from build123d import *

# Parameters (mm, degrees)
SKETCH_1_W          = 40
SKETCH_1_H          = 20
SKETCH_1_R          = 2.25
EXTRUDE_1_DEPTH     = 10
SKETCH_3_R          = 1.65
CUT_EXTRUDE_1_DEPTH = 11.5
CUT_EXTRUDE_START   = -11.5
SKETCH_4_R          = 1.65
CUT_EXTRUDE_2_DEPTH = 11.5


with BuildPart() as part:
    # 草图1 → 凸台-拉伸1 (new body)
    with BuildSketch(Plane.XY):
        with Locations((0.651465798, 0.195439739)):
            Rectangle(SKETCH_1_W, SKETCH_1_H)
        with Locations((-9.348534202, 0.195439739)):
            Circle(SKETCH_1_R, mode=Mode.SUBTRACT)
        with Locations((10.651465798, 0.195439739)):
            Circle(SKETCH_1_R, mode=Mode.SUBTRACT)
    extrude(amount=EXTRUDE_1_DEPTH)

    # 草图3 → 切除-拉伸1 (cut)
    with BuildSketch(Plane.ZY.offset(19.348534202)):
        with Locations(Location((5, 4.195439739, 0), (0, 0, 270))):
            Circle(SKETCH_3_R)
        with Locations(Location((5, -3.804560261, 0), (0, 0, 270))):
            Circle(SKETCH_3_R)
    extrude(amount=-CUT_EXTRUDE_1_DEPTH, mode=Mode.SUBTRACT)

    # 草图4 → 切除-拉伸2 (cut)
    with BuildSketch(Plane(origin=(20.651465798, 0, 0), x_dir=(0, 0, -1), z_dir=(1, 0, 0)).offset(CUT_EXTRUDE_START)):
        with Locations(Location((-5, 4.195439739, 0), (0, 0, 270))):
            Circle(SKETCH_4_R)
        with Locations(Location((-5, -3.804560261, 0), (0, 0, 270))):
            Circle(SKETCH_4_R)
    extrude(amount=CUT_EXTRUDE_2_DEPTH, mode=Mode.SUBTRACT)


solid = part.part
Geometry check sheet. Reference: the model listing, model coordinates, mm. A direction names the side the tool comes from. Give positions to 0.01 mm unless a question says otherwise; leave off trailing zeros. Write each loop counter-clockwise with the first axis right and the second up, starting at its lowest first coordinate (ties: lowest second). Pieces come first, ordered by that corner, then holes.
1) Go/stop test with flat-tipped pins: pin 1 Ø2.5 at (y, z) = (-4, 5) entering from -X; pin 2 Ø1.6 at (y, z) = (-4, 4.5) entering from +X. Record where each tip stops, or that it passes through.
Values follow:
pin 1: stops at x = -7.85
pin 2: stops at x = 9.15
2) Release check for a two-part mould opening along Z. For faces 4 (the face through (-11.596, 0.294, 4.93)), 5 (the face through (0, 0, 0)), 6 (the face through (-13.679, 5.505, 3.996)) record: released by +Z, released by -Z, zero draft, split by the parting line, or undercut.
Values follow:
face 4: zero draft
face 5: released by -Z
face 6: undercut
3) Thickness scan on line 1 (Y direction, x = 15.75, z = 5); line 2 (X direction, y = 0, z = 2.25); line 3 (X direction, y = -1.5, z = 6.75). Record the ranges inside material, lowest first.
Values follow:
line 1: y = -9.8 to -5.45, -2.15 to 2.55, 5.85 to 10.2
line 2: x = -19.35 to -11.59, -7.11 to 8.41, 12.89 to 20.65
line 3: x = -19.35 to -10.83, -7.87 to 9.17, 12.13 to 20.65
4) Set-up check for faces 1 (the face through (20.651, 0, 5)), 2 (the face through (-13.7, -3.4, 3.4)), 3 (the face through (14.8, -3.4, 6.6)): record each of +Z, -Z, +X, -X, +Y, -Y from which the full face is reachable in a straight line by a thin tool's end or side.
Values follow:
face 1: +Z, -Z, +X, +Y, -Y
face 2: -X
face 3: +X
5) Cross-section at C-C (z = 2). Record the boundary of the cut face in (x, y).
Values follow:
outline: (-19.35, -9.8) - (20.65, -9.8) - (20.65, 10.2) - (-19.35, 10.2) - close; hole circle Ø4.5 at (-9.35, 0.2); hole circle Ø4.5 at (10.65, 0.2)
6) Cross-section at A-A (x = 10.5). Record the boundary of the cut face in (y, z), plus the area to 3 significant figures.
Values follow:
outline: (-9.8, 0) - (-2.05, 0) - (-2.05, 10) - (-9.8, 10) - close; (2.44, 0) - (10.2, 0) - (10.2, 10) - (2.44, 10) - close; hole circle Ø3.3 at (-3.8, 5); hole circle Ø3.3 at (4.2, 5)
area: 138 mm2
7) Cross-section at B-B (z = 5.75). Record the boundary of the cut face in (x, y).
Values follow:
outline: (-19.35, -9.8) - (20.65, -9.8) - (20.65, -5.27) - (9.15, -5.27) - (9.15, -2.33) - (20.65, -2.33) - (20.65, 2.73) - (9.15, 2.73) - (9.15, 5.67) - (20.65, 5.67) - (20.65, 10.2) - (-19.35, 10.2) - (-19.35, 5.67) - (-7.85, 5.67) - (-7.85, 2.73) - (-19.35, 2.73) - (-19.35, -2.33) - (-7.85, -2.33) - (-7.85, -5.27) - (-19.35, -5.27) - close; hole circle Ø4.5 at (-9.35, 0.2); hole circle Ø4.5 at (10.65, 0.2)
